from build123d import *

# Parameters (mm, degrees)
CUT_EXTRUDE_1_DEPTH = 10


with BuildPart() as part:
    # 草图1 → 旋转1 (revolve)
    with BuildSketch(Plane.XY, mode=Mode.PRIVATE) as revolve_1_sk:
        Polygon((0, 7.958333333), (0, 6), (0.947, 5.053), (9.053, 5.053), (10, 6), (10, 11.875), (1.461538462, 11.875), align=None)
    revolve(revolve_1_sk.sketch.rotate(Axis((10, 0, 0), (-1, 0, 0)), 270), axis=Axis((10, 0, 0), (-1, 0, 0)))

    # 草图2 → 切除-拉伸1 (cut)
    with BuildSketch(Plane(origin=(0, 0, 0), x_dir=(0, 0, -1), z_dir=(1, 0, 0))):
        Polygon((-19, 10.969655115), (-19, -10.969655115), (0, -21.939310229), (19, -10.969655115), (19, 10.969655115), (0, 21.939310229), align=None)
        Polygon((-9.5, 5.484827557), (-9.5, -5.484827557), (0, -10.969655115), (9.5, -5.484827557), (9.5, 5.484827557), (0, 10.969655115), align=None, mode=Mode.SUBTRACT)
    extrude(amount=CUT_EXTRUDE_1_DEPTH, mode=Mode.SUBTRACT)


solid = part.part
The listing builds one solid part. Answer for the finished solid, in the listing's coordinates (mm). Round coordinates to 2 decimals unless told otherwise and drop trailing zeros. Order: outer loops, then holes, each group sorted by start corner. A loop starts at its lowest first (then second) coordinate and runs counter-clockwise, first axis right, second up. Notation, with made-up numbers: (31.25, -33) - (41.25, -33) arc R11 ccw to (41.25, -29) - close; hole circle Ø4 at (-12.75, 26). An arc over 180 degrees is marked (long way). Write item = value, one per line. Start each with the question number.
1) Straight lines are drawn through the part: L1, parallel to Z at x = 7.25, y = 4.5; L2, parallel to Z at x = 9, y = 1.5; L3, parallel to Y at x = 9.25, z = -4. For each, find the intervals that lie inside material, in ascending order.
2) Section A-A, the plane x = 7.5 is taken. Write down the section's boundary in (y, z).
3) Given pin 1 (6 mm diameter, centred on x = 3, y = -7.5, fed in from +Z); pin 2 (9 mm diameter, centred on y = 0, z = 0, fed in from -X), each flat-ended and moving along its own axis, determine where each tip first touches the part or whether it passes through.
4) Section B-B, the plane y = 0 is taken. Write down the section's boundary in (x, z), plus the area to 3 significant figures.
5) For a pull along Y with two mould halves and no side action, classify faces 1 (the flat face through (5.2, 8.2, -4.8)), 2 (the cylindrical face through (5.06, 3.42, -3.72)), 3 (the flat face through (5, 0, -9.5)), 4 (the flat face through (5.222, -8.266, -4.684)) as released by +Y, released by -Y, zero draft, split by the parting line, or undercut.
Results list:
q1.L1 = -9.5 to -2.3, 2.3 to 9.5
q1.L2 = -9.5 to -4.83, 4.83 to 9.5
q1.L3 = -8.66 to -3.4, 3.4 to 8.66
q2.outline = (-10.97, 0) - (-5.48, -9.5) - (5.48, -9.5) - (10.97, 0) - (5.48, 9.5) - (-5.48, 9.5) - close; hole circle Ø10.11 at (0, 0)
q3.pin_1 = 9.5
q3.pin_2 = through
q4.outline = (0, -7.96) - (0.58, -9.5) - (10, -9.5) - (10, -6) - (9.05, -5.05) - (0.95, -5.05) - (0, -6) - close; (0, 6) - (0.95, 5.05) - (9.05, 5.05) - (10, 6) - (10, 9.5) - (0.58, 9.5) - (0, 7.96) - close
q4.area = 86.3 mm^2
q5.face_1 = released by +Y
q5.face_2 = undercut
q5.face_3 = zero draft
q5.face_4 = released by -Y
